```python
from build123d import *

# Parameters (mm, degrees)
SKETCH_1_W               = 110
SKETCH_1_H               = 90
EXTRUDE_1_DEPTH          = 15
CUT_EXTRUDE_1_DEPTH      = 73.629195232
CUT_EXTRUDE_1_DEPTH_BACK = 73.629195232
SKETCH_2_W               = 13.2
SKETCH_2_H               = 11.9
CUT_EXTRUDE_2_DEPTH      = 73.629195232
HOLE_WIZARD_M5_1_D       = 4.2
HOLE_WIZARD_M5_1_DEPTH   = 12.4
HOLE_WIZARD_M5_1_TIP     = 1.2618073
CHAMFER_1_SIZE           = 0.5


with BuildPart() as part:
    # 草图1 → 凸台-拉伸1 (new body)
    with BuildSketch(Plane.XY):
        Rectangle(SKETCH_1_W, SKETCH_1_H)
    extrude(amount=EXTRUDE_1_DEPTH)

    # 草图2 → 切除-拉伸1 (cut, two sides: drawn at the far end of the back side and taken through both)
    with BuildSketch(Plane.XY.offset(15).offset(-CUT_EXTRUDE_1_DEPTH_BACK)):
        with Locations((0, 39.05)):
            Rectangle(SKETCH_2_W, SKETCH_2_H)
    extrude(amount=CUT_EXTRUDE_1_DEPTH + CUT_EXTRUDE_1_DEPTH_BACK, mode=Mode.SUBTRACT)

    # 草图3 → 切除-拉伸2 (cut, through all)
    with BuildSketch(Plane.XY.offset(15)):
        with BuildLine():
            Line((-12.5, 37.15), (12.5, 37.15))
            ThreePointArc((12.5, 37.15), (14.525, 35.125), (12.5, 33.1))
            Line((12.5, 33.1), (-12.5, 33.1))
            ThreePointArc((-12.5, 33.1), (-14.525, 35.125), (-12.5, 37.15))
        make_face()
    extrude(amount=-CUT_EXTRUDE_2_DEPTH, mode=Mode.SUBTRACT)

    # M5 螺纹孔1
    with Locations(Plane(origin=(0, -45, 0), x_dir=(-1, 0, 0), z_dir=(0, -1, 0))):
        with Locations((-47.5, -7.5), (47.5, -7.5)):
            Hole(HOLE_WIZARD_M5_1_D / 2, depth=HOLE_WIZARD_M5_1_DEPTH)
            with Locations((0, 0, -(HOLE_WIZARD_M5_1_DEPTH + HOLE_WIZARD_M5_1_TIP / 2))):  # 118° drill point
                Cone(0, HOLE_WIZARD_M5_1_D / 2, HOLE_WIZARD_M5_1_TIP, mode=Mode.SUBTRACT)

    # 倒角1
    chamfer_1_edges = [part.edges().sort_by_distance(p)[0] for p in [
        (-55, 0, 15),
        (-30.8, 45, 0),
        (-30.8, 45, 15),
        (0, -45, 15),
        (-6.6, 45, 7.5),
        (6.6, 45, 7.5),
        (55, 0, 15),
        (0, -45, 0),
        (-55, 0, 0),
        (30.8, 45, 0),
        (55, 0, 0),
        (55, -45, 7.5),
        (-55, -45, 7.5),
        (-55, 45, 7.5),
        (55, 45, 7.5),
        (30.8, 45, 15),
    ]]
    chamfer(chamfer_1_edges, length=CHAMFER_1_SIZE)


solid = part.part
```
Source: CAD feature listing. Evaluate the final solid. Frame: model axes, mm. A direction names the side the tool comes from. Coordinates: 2 decimals unless noted, no trailing zeros. Loops run counter-clockwise (first coordinate to the right, second up) from the corner with the lowest first, then second, coordinate; pieces in that order, holes last. Notation, with made-up numbers: M 3,76 L 62,76 A21 ccw 62,111 Z; hole C 6,6 d2. An arc over 180 degrees is marked long. Put each result on its own line as item: value. Start each with the question number.
1) Reachability of faces 1 (the face through (48.63, -38.71, 5.73)), 2 (the face through (10, 37.15, 8)), 3 (the face through (-6.6, 41, 7)) from +Z, -Z, +X, -X, +Y, -Y: full face, straight path, thin tool, end or side. Return the list, or none.
2) Cut plane A-A on z = 12.25. Return the cut outline in (x, y) (3 decimals).
3) Ray query, L1, parallel to Z at x = 47.5, y = -36.25; L2, parallel to X at y = -40, z = 8.5; L3, parallel to Y at x = -9, z = 12. Return the intervals inside material, ascending. Write a range as from..to.
4) Contact query for a flat-ended pin moving along its axis: pin 1 Ø5.5 at (x, z) = (47.5, 7.5) entering from -Y. Output: stop coordinate, or through.
5) Pull-direction query (X, two-part tool) for faces 4 (the face through (-55, -1, 7)), 5 (the face through (0, 33.1, 8)), 6 (the face through (55, -1, 7)), 7 (the face through (14.525, 35.17, 7.605)); classes: pulls with the +X half, pulls with the -X half, needs draft (parallel to the pull), parting line crosses it, or undercut.
The answers:
1. face 1: -Y
1. face 2: +Z, -Z
1. face 3: +Z, -Z, +Y
2. outline: M -55,-44.5 L -54.5,-45 L 54.5,-45 L 55,-44.5 L 55,44.5 L 54.5,45 L 7.1,45 L 6.6,44.5 L 6.6,37.15 L 12.5,37.15 A2.025 cw 12.5,33.1 L -12.5,33.1 A2.025 cw -12.5,37.15 L -6.6,37.15 L -6.6,44.5 L -7.1,45 L -54.5,45 L -55,44.5 Z
3. L1: z = 0..5.4, 9.6..15
3. L2: x = -55..-49.35, -45.65..45.65, 49.35..55
3. L3: y = -45..33.1, 37.15..45
4. pin 1: stops at y = -45
5. face 4: pulls with the -X half
5. face 5: undercut
5. face 6: pulls with the +X half
5. face 7: undercut
